```python
from build123d import *

# Parameters (mm, degrees)
SKETCH_1_W             = 60
SKETCH_1_H             = 90
SKETCH_1_R             = 20
EXTRUDE_1_DEPTH        = 7
EXTRUDE_START          = -2
SKETCH_2_R             = 20
SKETCH_2_R_2           = 18.5
EXTRUDE_2_DEPTH        = 2
CHAMFER_1_SIZE         = 10
HOLE_WIZARD_M6_1_D     = 5
HOLE_WIZARD_M6_1_DEPTH = 14
HOLE_WIZARD_M6_1_TIP   = 1.502151548


with BuildPart() as part:
    # 草图1 → 凸台-拉伸1 (new, symmetric)
    with BuildSketch(Plane.XY):
        Rectangle(SKETCH_1_W, SKETCH_1_H)
        with Locations((0, 15)):
            Circle(SKETCH_1_R, mode=Mode.SUBTRACT)
    extrude(amount=EXTRUDE_1_DEPTH, both=True)

    # 草图2 → 凸台-拉伸2 (add)
    with BuildSketch(Plane.XY.offset(7).offset(EXTRUDE_START)):
        with Locations((0, 15)):
            Circle(SKETCH_2_R)
        with Locations((0, 15)):
            Circle(SKETCH_2_R_2, mode=Mode.SUBTRACT)
    extrude(amount=EXTRUDE_2_DEPTH)

    # 倒角1
    chamfer_1_edges = [part.edges().sort_by_distance(p)[0] for p in [
        (-30, 45, 0),
        (30, 45, 0),
    ]]
    chamfer(chamfer_1_edges, length=CHAMFER_1_SIZE)

    # M6 螺纹孔1
    with Locations(Plane(origin=(-24, -45, 0), x_dir=(0, 0, -1), z_dir=(0, -1, 0))):
        with Locations((0, 0), (0, 48)):
            Hole(HOLE_WIZARD_M6_1_D / 2, depth=HOLE_WIZARD_M6_1_DEPTH)
            with Locations((0, 0, -(HOLE_WIZARD_M6_1_DEPTH + HOLE_WIZARD_M6_1_TIP / 2))):  # 118° drill point
                Cone(0, HOLE_WIZARD_M6_1_D / 2, HOLE_WIZARD_M6_1_TIP, mode=Mode.SUBTRACT)


solid = part.part
```
Read the model definition and answer for the solid it produces. Units are mm, in the model's axes. A direction names the side the tool comes from. Coordinates: 2 decimals unless noted, no trailing zeros. Write each loop counter-clockwise with the first axis right and the second up, starting at its lowest first coordinate (ties: lowest second). Pieces come first, ordered by that corner, then holes. Notation, with made-up numbers: (-33, 86) -> (4, 86) arc R26 ccw to (4, 116) -> close; hole circle Ø1 at (-27.5, 81.25). An arc over 180 degrees is marked (long way). Answer as a JSON object with one key per item and string values.
Q1. A tool of negligible diameter and unlimited length cuts with its end or side. For faces 4 (the cylindrical face through (-21.52, -37.9, -0.33)), 5 (the flat face through (25, 40, 0)), 6 (the flat face through (6, -3, 5)), from which of +Z, -Z, +X, -X, +Y, -Y can it reach the whole face along a straight path? Write none if from no direction.
The answers:
{"face 4": "-Y", "face 5": "+Z, -Z, +X, +Y", "face 6": "-Z"}
Q2. Flat-ended cylindrical pins translate along their axes: pin 1 Ø22 at (x, y) = (0, 15) entering from +Z; pin 2 Ø3 at (x, z) = (-24, 0) entering from +Y. Find the tip coordinate at first contact, or state that the pin passes through.
The answers:
{"pin 1": "passes through", "pin 2": "stops at y = 42.5"}
Q3. The part is cut by section C-C on y = 15. Give the vertices of the cut face in (x, z).
The answers:
{"outline": "(-30, -7) -> (-20, -7) -> (-20, 5) -> (-18.5, 5) -> (-18.5, 7) -> (-30, 7) -> close; (18.5, 5) -> (20, 5) -> (20, -7) -> (30, -7) -> (30, 7) -> (18.5, 7) -> close"}
Q4. Determine the mould class of faces 1 (the flat face through (0, 45, 0)), 2 (the cylindrical face through (26.48, -37.9, -0.33)), 3 (the flat face through (0, -9, -7)) for opening direction Z: pulls with the +Z half, pulls with the -Z half, needs draft (parallel to the pull), parting line crosses it, or undercut.
The answers:
{"face 1": "needs draft", "face 2": "undercut", "face 3": "pulls with the -Z half"}
Q5. The part is cut by section B-B on x = 0. Give the vertices of the cut face in (y, z).
The answers:
{"outline": "(-45, -7) -> (-5, -7) -> (-5, 5) -> (-3.5, 5) -> (-3.5, 7) -> (-45, 7) -> close; (33.5, 5) -> (35, 5) -> (35, -7) -> (45, -7) -> (45, 7) -> (33.5, 7) -> close"}
Q6. Consider line 1 (X direction, y = -42, z = 0); line 2 (Z direction, x = -24, y = -37); line 3 (Y direction, x = 0.5, z = 3.75). Determine where each line is inside the solid, lowest interval first. Write a range as [from, to].
The answers:
{"line 1": "x = [-30, -26.5], [-21.5, 21.5], [26.5, 30]", "line 2": "z = [-7, -2.5], [2.5, 7]", "line 3": "y = [-45, -4.99], [34.99, 45]"}
Q7. The part is cut by section A-A on z = 3.5. Give the vertices of the cut face in (x, y), then the cut area to 3 significant figures.
The answers:
{"outline": "(-30, -45) -> (30, -45) -> (30, 35) -> (20, 45) -> (-20, 45) -> (-30, 35) -> close; hole circle Ø40 at (0, 15)", "area": "4,040 mm2"}
Q8. The part is cut by section D-D on y = -39. Give the vertices of the cut face in (x, z), then the cut area to 3 significant figures.
The answers:
{"outline": "(-30, -7) -> (30, -7) -> (30, 7) -> (-30, 7) -> close; hole circle Ø5 at (-24, 0); hole circle Ø5 at (24, 0)", "area": "801 mm2"}
